Can you work these out from the drawing? Everything is in mm from the part's minimum corner. A direction names the side the tool comes from. Give positions to 0.01 mm unless a question says otherwise; leave off trailing zeros. Order: outer loops, then holes, each group sorted by start corner. A loop starts at its lowest first (then second) coordinate and runs counter-clockwise, first axis right, second up. Notation, with made-up numbers: (-18, -37) - (7, -37) arc R37 ccw to (7, 2) - close; hole circle Ø9 at (74.25, -19). An arc over 180 degrees is marked (long way). Answer as a JSON object with one key per item and string values.
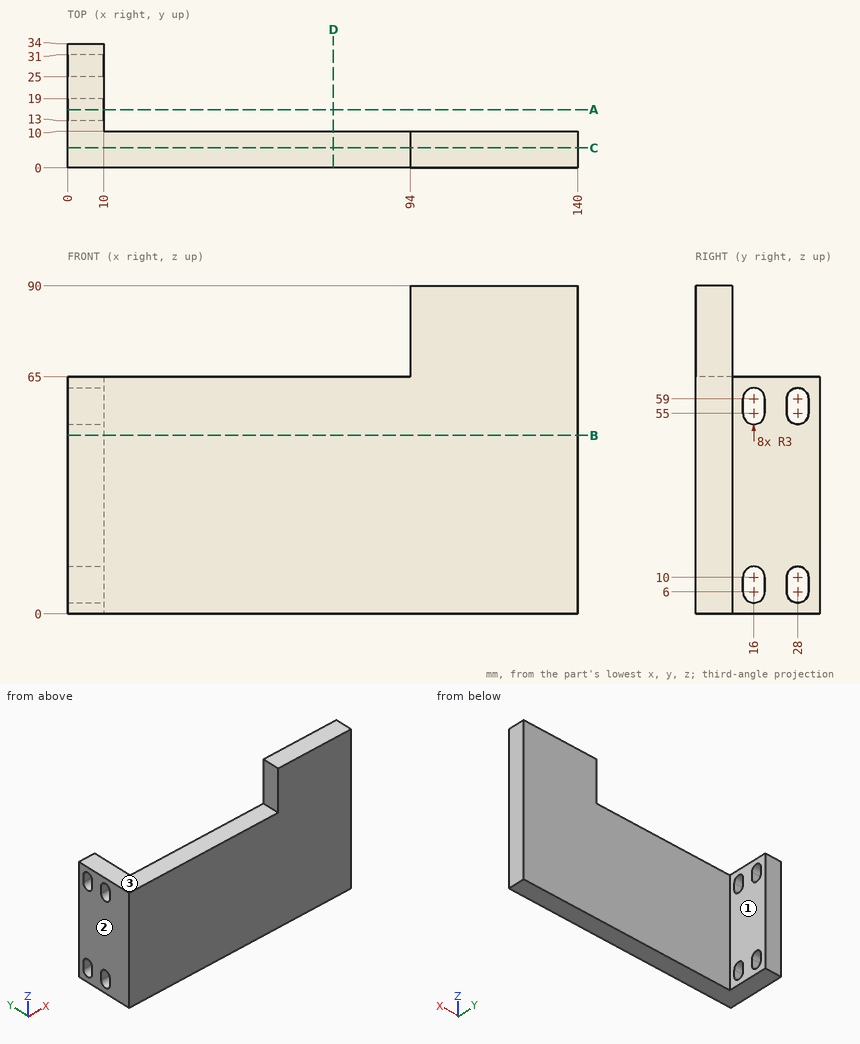
Q1. Which directions (+Z, -Z, +X, -X, +Y, -Y) give clear straight access to the entire face, cutting with the end or side of a thin tool? Please do the marked faces 1, 2 and 3.
Recorded:
{"face 1": "+Z, -Z, +X, +Y", "face 2": "+Z, -Z, -X, +Y, -Y", "face 3": "+Z, -X, +Y, -Y"}
Q2. I need wall thicknesses on L1, parallel to Z at x = 28, y = 2; L2, parallel to Y at x = 133, z = 56. Which ranges of each line are inside material? Lowest first, please.
Recorded:
{"L1": "z = 0 to 65", "L2": "y = 0 to 10"}
Q3. If we section it at D-D, the plane x = 73: Please give me the cut outline in (y, z), then the cut area to 3 significant figures.
Recorded:
{"outline": "(0, 0) - (10, 0) - (10, 65) - (0, 65) - close", "area": "650 mm^2"}
Q4. If we section it at A-A, the plane y = 16: Please give me the cut outline in (x, z), then the cut area to 3 significant figures.
Recorded:
{"outline": "(0, 0) - (10, 0) - (10, 3) - (0, 3) - close; (0, 13) - (10, 13) - (10, 52) - (0, 52) - close; (0, 62) - (10, 62) - (10, 65) - (0, 65) - close", "area": "450 mm^2"}
Q5. If we section it at C-C, the plane y = 5.5: Please give me the cut outline in (x, z), then the cut area to 4 significant figures.
Recorded:
{"outline": "(0, 0) - (140, 0) - (140, 90) - (94, 90) - (94, 65) - (0, 65) - close", "area": "10,250 mm^2"}
Q6. If we section it at B-B, the plane z = 49: Please give me the cut outline in (x, y), then the cut area to 3 significant figures.
Recorded:
{"outline": "(0, 0) - (140, 0) - (140, 10) - (10, 10) - (10, 34) - (0, 34) - close", "area": "1,640 mm^2"}
Q7. I'm going to push flat-ended pins straight in: pin 1 Ø1.2 at (x, z) = (3.5, 57) entering from -Y; pin 2 Ø10 at (x, y) = (27.5, 19.5) entering from +Z; pin 3 Ø6 at (x, z) = (98, 74.5) entering from +Y; pin 4 Ø8 at (y, z) = (5.5, 77) entering from -X. Where does each tip first touch, or does it pass through?
Recorded:
{"pin 1": "stops at y = 0", "pin 2": "passes through", "pin 3": "stops at y = 10", "pin 4": "stops at x = 94"}
